Part model, mm, in its own coordinate system. A direction names the side the tool comes from. Give positions to 0.01 mm unless a question says otherwise; leave off trailing zeros. Order: outer loops, then holes, each group sorted by start corner. A loop starts at its lowest first (then second) coordinate and runs counter-clockwise, first axis right, second up.
from build123d import *

# Parameters (mm, degrees)
SKETCH_1_R      = 1.25
EXTRUDE_1_DEPTH = 1.2


with BuildPart() as part:
    # 草图1 → 凸台-拉伸1 (new body)
    with BuildSketch(Plane.XY):
        with BuildLine():
            Line((5.426958413, -13.101836603), (6.582155037, -15.890727959))
            ThreePointArc((6.582155037, -15.890727959), (0, 17.2), (-6.582155037, -15.890727959))
            Line((-6.582155037, -15.890727959), (-5.426958413, -13.101836603))
            ThreePointArc((-5.426958413, -13.101836603), (-6.278083953, -10.114718223), (-9.380614428, -10.261672481))
            ThreePointArc((-9.380614428, -10.261672481), (-10.498981278, -10.625780527), (-11.536197995, -10.071253196))
            ThreePointArc((-11.536197995, -10.071253196), (0, 14), (11.536197995, -10.071253196))
            ThreePointArc((11.536197995, -10.071253196), (10.498981278, -10.625780527), (9.380614428, -10.261672481))
            ThreePointArc((9.380614428, -10.261672481), (6.278083953, -10.114718223), (5.426958413, -13.101836603))
        make_face()
        with Locations(Location((-7.736657244, -12.145128022, 0), (0, 0, 180))):
            Circle(SKETCH_1_R, mode=Mode.SUBTRACT)
        with Locations(Location((7.736657244, -12.145128022, 0), (0, 0, 180))):
            Circle(SKETCH_1_R, mode=Mode.SUBTRACT)
    extrude(amount=-EXTRUDE_1_DEPTH)


solid = part.part
Item 1: Pull direction X, two halves, no side cores. Call faces 1 (the face through (0.662, 17.187, -0.592)), 2 (the face through (-1.4, 14.2, -1.2)), 3 (the face through (0, 14, -1)): released by +X, released by -X, zero draft, split by the parting line, or undercut.
Item 2: Band-saw the part on B-B on z = -0.8. List the corners of the cut face in (x, y), plus the area to 3 significant figures.
Item 3: Which spindle directions (+Z, -Z, +X, -X, +Y, -Y) get a long thin tool onto all of the face, cutting with end or side? Do faces 4 (the face through (-6.013, -14.516, -0.592)), 5 (the face through (-1.4, 14.2, 0)), 6 (the face through (10.516, -10.624, -0.592)). Say none if no direction does.
Item 4: Drill centre lines: probe 1 along X at (y, z) = (-10, -0.05); probe 2 along X at (y, z) = (3, -0.6); probe 3 along Y at (x, z) = (-7.5, -0.15). Where is each one in solid material? Low to high.
Item 5: Band-saw the part on D-D on x = 13. List the corners of the cut face in (y, z).
Item 6: Band-saw the part on A-A on y = 3.5. List the corners of the cut face in (x, z), plus the area to 3 significant figures.
Item 7: Band-saw the part on C-C on x = -8.5. List the corners of the cut face in (y, z).
Working result:
1. face 1: split by the parting line
1. face 2: zero draft
1. face 3: undercut
2. outline: (-11.54, -10.07) arc R14.8 cw (long way) to (11.54, -10.07) arc R1.5 cw to (9.38, -10.26) arc R2.5 ccw to (5.43, -13.1) - (6.58, -15.89) arc R17.2 ccw (long way) to (-6.58, -15.89) - (-5.43, -13.1) arc R2.5 ccw to (-9.38, -10.26) arc R1.5 cw to start; hole circle Ø2.5 at (-7.74, -12.15); hole circle Ø2.5 at (7.74, -12.15)
2. area: 242 mm2
3. face 4: +Z, -Z, -Y
3. face 5: +Z, +X, -X, +Y, -Y
3. face 6: +Z, -Z
4. probe 1: x = -13.99 to -11.59, -9.02 to -6.45, 6.45 to 9.02, 11.59 to 13.99
4. probe 2: x = -16.94 to -14.3, 14.3 to 16.94
4. probe 3: y = -15.48 to -13.37, -10.92 to -9.66, 11.96 to 15.48
5. outline: (-11.26, -1.2) - (-7.87, -1.2) - (-7.87, 0) - (-11.26, 0) - close; (6.27, -1.2) - (11.26, -1.2) - (11.26, 0) - (6.27, 0) - close
6. outline: (-16.84, -1.2) - (-14.16, -1.2) - (-14.16, 0) - (-16.84, 0) - close; (14.16, -1.2) - (16.84, -1.2) - (16.84, 0) - (14.16, 0) - close
6. area: 6.43 mm2
7. outline: (-14.95, -1.2) - (-13.13, -1.2) - (-13.13, 0) - (-14.95, 0) - close; (-11.16, -1.2) - (-9.76, -1.2) - (-9.76, 0) - (-11.16, 0) - close; (11.32, -1.2) - (14.95, -1.2) - (14.95, 0) - (11.32, 0) - close
